Geometry check sheet. Reference: the model listing, model coordinates, mm. A direction names the side the tool comes from. Coordinates: 2 decimals unless noted, no trailing zeros. Write each loop counter-clockwise with the first axis right and the second up, starting at its lowest first coordinate (ties: lowest second). Pieces come first, ordered by that corner, then holes. Notation, with made-up numbers: (61, -5) -> (89, -5) arc R25 cw to (89, 12) -> close; hole circle Ø9 at (-32.5, 41.5). An arc over 180 degrees is marked (long way). Put each result on its own line as item: value. Start each with the question number.
from build123d import *

# Parameters (mm, degrees)
FLANGE_PROFILE_90_R        = 45
FLANGE_90_DEPTH            = 14.2
FLANGE_HOLES_SKETCH_R      = 6.25
FLANGE_HOLES_4X_12_5_DEPTH = 14.2
SHANK_PROFILE_40_R         = 20
SHANK_40_DEPTH             = 44.2
BORE_PROFILE_30_R          = 15
THROUGH_BORE_30_DEPTH      = 87.374533284
BORE_CHAMFER_3MM_SIZE      = 3
BORE_CHAMFER_3MM_SIZE2     = 0.18348786
COLLAR_PROFILE_50_38_R     = 25
COLLAR_PROFILE_50_38_R_2   = 19
END_COLLAR_50_DEPTH        = 30
FLANGE_EDGE_FILLET_R2_R    = 2
FLANGE_SHANK_FILLET_R2_R   = 2
COLLAR_FILLET_R2_A_R       = 2
SHANK_BORE_FILLET_R2_R     = 2
COLLAR_FILLET_R2_B_R       = 2


with BuildPart() as part:
    # Flange Profile Ø90 → Flange Ø90 (new body)
    with BuildSketch(Plane.XY):
        Circle(FLANGE_PROFILE_90_R)
    extrude(amount=FLANGE_90_DEPTH)

    # Flange Holes Sketch → Flange Holes 4xØ12.5 (cut)
    with BuildSketch(Plane.XY.offset(14.2)):
        with Locations((0, 32.5)):
            Circle(FLANGE_HOLES_SKETCH_R)
        with Locations((0, -32.5)):
            Circle(FLANGE_HOLES_SKETCH_R)
        with Locations((-32.5, 0)):
            Circle(FLANGE_HOLES_SKETCH_R)
        with Locations((32.5, 0)):
            Circle(FLANGE_HOLES_SKETCH_R)
    extrude(amount=-FLANGE_HOLES_4X_12_5_DEPTH, mode=Mode.SUBTRACT)

    # Shank Profile Ø40 → Shank Ø40 (add)
    with BuildSketch(Plane.XY.offset(14.2)):
        Circle(SHANK_PROFILE_40_R)
    extrude(amount=SHANK_40_DEPTH)

    # Bore Profile Ø30 → Through Bore Ø30 (cut, through all)
    with BuildSketch(Plane(origin=(0, 0, 0), x_dir=(-1, 0, 0), z_dir=(0, 0, -1))):
        Circle(BORE_PROFILE_30_R)
    extrude(amount=-THROUGH_BORE_30_DEPTH, mode=Mode.SUBTRACT)

    # Bore Chamfer 3mm
    bore_chamfer_3mm_edges = [part.edges().sort_by_distance(p)[0] for p in [
        (15, 0, 0),
    ]]
    bore_chamfer_3mm_side = [part.faces().sort_by_distance(p)[0] for p in [
        (-43.727207794, 0, 0),
    ]]
    chamfer(bore_chamfer_3mm_edges, length=BORE_CHAMFER_3MM_SIZE, length2=BORE_CHAMFER_3MM_SIZE2, reference=bore_chamfer_3mm_side[0])

    # Collar Profile Ø50-Ø38 → End Collar Ø50 (add)
    with BuildSketch(Plane.XY.offset(58.4)):
        Circle(COLLAR_PROFILE_50_38_R)
        Circle(COLLAR_PROFILE_50_38_R_2, mode=Mode.SUBTRACT)
    extrude(amount=END_COLLAR_50_DEPTH)

    # Flange Edge Fillet R2
    flange_edge_fillet_r2_edges = [part.edges().sort_by_distance(p)[0] for p in [
        (-45, 0, 14.2),
    ]]
    fillet(flange_edge_fillet_r2_edges, radius=FLANGE_EDGE_FILLET_R2_R)

    # Flange-Shank Fillet R2
    flange_shank_fillet_r2_edges = [part.edges().sort_by_distance(p)[0] for p in [
        (-20, 0, 14.2),
    ]]
    fillet(flange_shank_fillet_r2_edges, radius=FLANGE_SHANK_FILLET_R2_R)

    # Collar Fillet R2 A
    collar_fillet_r2_a_edges = [part.edges().sort_by_distance(p)[0] for p in [
        (-19, 0, 88.4),
    ]]
    fillet(collar_fillet_r2_a_edges, radius=COLLAR_FILLET_R2_A_R)

    # Shank Bore Fillet R2
    shank_bore_fillet_r2_edges = [part.edges().sort_by_distance(p)[0] for p in [
        (15, 0, 58.4),
    ]]
    fillet(shank_bore_fillet_r2_edges, radius=SHANK_BORE_FILLET_R2_R)

    # Collar Fillet R2 B
    collar_fillet_r2_b_edges = [part.edges().sort_by_distance(p)[0] for p in [
        (-25, 0, 58.4),
    ]]
    fillet(collar_fillet_r2_b_edges, radius=COLLAR_FILLET_R2_B_R)


solid = part.part
Item 1: Section check D-D, the plane z = 66. Enter the section's corners in (x, y), and give its area (3 significant figures).
Item 2: Scan lines: line 1 along Y through (x, z) = (0, 9); line 2 along Z through (x, y) = (7.5, -22); line 3 along Y through (x, z) = (0, 67). Record each from-to range of solid material in increasing order. Write a range as [from, to].
Item 3: Section check B-B, the plane x = 0. Give the number of separate pieces and of enclosed holes in the cut face, and give its area (3 significant figures).
Item 4: Section check A-A, the plane z = 37.5. Enter the section's corners in (x, y).
Item 5: Mould release check, pull along Y, two halves, no side actions. Record for faces 1 (the cylindrical face through (-0.8, 38.7, 7.2)), 2 (the cylindrical face through (20.765, -39.923, 6.015)), 3 (the flat face through (-7, 19, 58.4)): released by +Y, released by -Y, zero draft, split by the parting line, or undercut.
Item 6: Go/stop test with flat-tipped pins: P1, Ø6, axis at y = 23.5, z = 65.5, coming from the +X side; P2, Ø3, axis at x = 17, z = 64, coming from the +Y side; P3, Ø1, axis at x = 13.5, z = 55.5, coming from the -Y side. Record where each tip stops, or that it passes through.
Item 7: Access from +Z, -Z, +X, -X, +Y, -Y to the whole of each face (thin tool, end or side, straight path). Record for faces 4 (the cylindrical face through (23.846, 7.509, 74.204)), 5 (the cylindrical face through (14.985, 0.66, 27.898)), 6 (the cylindrical face through (-4.336, -19.524, 37.005)).
From the geometry:
1. outline: circle Ø50 at (0, 0); hole circle Ø38 at (0, 0)
1. area: 829 mm²
2. line 1: [-45, -38.75], [-26.25, -15], [15, 26.25], [38.75, 45]
2. line 2: [0, 14.2], [58.41, 88.4]
2. line 3: [-25, -19], [19, 25]
3. separate pieces: 4
3. enclosed holes: 0
3. area: 1,290 mm²
4. outline: circle Ø40 at (0, 0); hole circle Ø30 at (0, 0)
5. face 1: undercut
5. face 2: split by the parting line
5. face 3: zero draft
6. P1: x = 14.31
6. P2: y = 19.62
6. P3: y = -15.2
7. face 4: +Z
7. face 5: +Z, -Z
7. face 6: none
